from build123d import *

# Parameters (mm, degrees)
SKETCH1_R           = 40
BOSS_EXTRUDE1_DEPTH = 16
CUT_EXTRUDE2_DEPTH  = 500


with BuildPart() as part:
    # Sketch1 → Boss-Extrude1 (new body)
    with BuildSketch(Plane.XY):
        with BuildLine():
            Line((0, 40), (0, 164))
            Line((0, 164), (489.6, 105))
            Line((489.6, 105), (489.6, 40))
            ThreePointArc((489.6, 40), (449.6, 0), (489.6, -40))
            Line((489.6, -40), (489.6, -105))
            Line((489.6, -105), (0, -164))
            Line((0, -164), (0, -40))
            ThreePointArc((0, -40), (40, 0), (0, 40))
        make_face()
        with Locations((241.4, 0)):
            Circle(SKETCH1_R, mode=Mode.SUBTRACT)
        with Locations((126.4, 88.333889345)):
            Circle(SKETCH1_R, mode=Mode.SUBTRACT)
        with Locations((356.4, 60.617386077)):
            Circle(SKETCH1_R, mode=Mode.SUBTRACT)
        with Locations((126.4, -88.333889345)):
            Circle(SKETCH1_R, mode=Mode.SUBTRACT)
        with Locations((356.4, -60.617386077)):
            Circle(SKETCH1_R, mode=Mode.SUBTRACT)
    extrude(amount=BOSS_EXTRUDE1_DEPTH)

    # Sketch3 → Cut-Extrude2 (cut, along a direction that is not the sketch's normal)
    with BuildSketch(Plane(origin=(19.480184067, -161.652510498, 0), x_dir=(0.9928172236743598, 0.11964096445422229, 0), z_dir=(0.11964096445422229, -0.9928172236743598, 0))):
        Polygon((473.521011443, 16), (464.021011443, 0), (473.521011443, 0), align=None)
        Polygon((-19.62111817, 16), (-19.62111817, 0), (13.87888183, 0), align=None)
    extrude(amount=-CUT_EXTRUDE2_DEPTH, dir=(0, -1, 0), mode=Mode.SUBTRACT)


solid = part.part
The listing builds one solid part. Answer for the finished solid, in the listing's coordinates (mm). Round coordinates to 2 decimals unless told otherwise and drop trailing zeros. Write each loop counter-clockwise with the first axis right and the second up, starting at its lowest first coordinate (ties: lowest second). Pieces come first, ordered by that corner, then holes. Notation, with made-up numbers: (18, -24.75) - (47, -24.75) arc R17 cw to (47, -9.75) - close; hole circle Ø3 at (9.25, 66.25). An arc over 180 degrees is marked (long way). Use one line per item in the form item = value. Start each with the question number.
Item 1: A cutting plane is placed at C-C (x = 356.4). Write down the section's boundary in (y, z).
Item 2: Determine the mould class of faces 1 (the flat face through (248.227, -134.087, 7.888)), 2 (the flat face through (17.05, -94.02, 7.8)), 3 (the flat face through (241.373, 134.913, 7.888)), 4 (the cylindrical face through (279.553, 12.015, 7.888)) for opening direction Y: +Y half, -Y half, draft (parallel to the pull), parting line (faces both ways), or undercut.
Item 3: Flat-ended cylindrical pins translate along their axes: pin 1 Ø3 at (y, z) = (-54.5, 10) entering from -X; pin 2 Ø5 at (x, z) = (75, 3) entering from -Y; pin 3 Ø1 at (y, z) = (-17, 6.5) entering from +X. Find the tip coordinate at first contact, or state that the pin passes through.
Item 4: A cutting plane is placed at B-B (y = -55.5). Write down the section's boundary in (x, z), plus the area to 3 significant figures.
Item 5: A cutting plane is placed at A-A (x = 269). Write down the section's boundary in (y, z), plus the area to 3 significant figures.
Item 6: Find the intervals of material crossed by line 1 (X direction, y = 73, z = 5.75); line 2 (X direction, y = -61, z = 10.5); line 3 (Y direction, x = 126.4, z = 4.25), in increasing order. Write a range as [from, to].
Item 7: A cutting plane is placed at D-D (z = 7.25). Write down the section's boundary in (x, y), plus the area to 3 significant figures.
The answers:
q1.outline = (-121.05, 0) - (-100.62, 0) - (-100.62, 16) - (-121.05, 16) - close; (-20.62, 0) - (20.62, 0) - (20.62, 16) - (-20.62, 16) - close; (100.62, 0) - (121.05, 0) - (121.05, 16) - (100.62, 16) - close
q2.face_1 = -Y half
q2.face_2 = draft
q2.face_3 = +Y half
q2.face_4 = undercut
q3.pin_1 = 9.35
q3.pin_2 = -155.26
q3.pin_3 = 453.63
q4.outline = (0, 16) - (33.26, 0) - (103.55, 0) - (103.55, 16) - close; (149.25, 0) - (316.73, 0) - (316.73, 16) - (149.25, 16) - close; (396.07, 0) - (480.17, 0) - (489.6, 16) - (396.07, 16) - close
q4.area = 5,490 mm^2
q5.outline = (-131.58, 0) - (-28.95, 0) - (-28.95, 16) - (-131.58, 16) - close; (28.95, 0) - (131.58, 0) - (131.58, 16) - (28.95, 16) - close
q5.area = 3,280 mm^2
q6.line_1 = [21.31, 89.46], [163.34, 318.36], [394.44, 483.56]
q6.line_2 = [11.43, 97.2], [155.6, 316.4], [396.4, 486.36]
q6.line_3 = [-148.77, -128.33], [-48.33, 48.33], [128.33, 148.77]
q7.outline = (18.19, -161.81) - (484.44, -105.62) - (484.44, -39.67) arc R40 cw to (484.44, 39.67) - (484.44, 105.62) - (18.19, 161.81) - (18.19, 35.63) arc R40 cw to (18.19, -35.63) - close; hole circle Ø80 at (126.4, -88.33); hole circle Ø80 at (126.4, 88.33); hole circle Ø80 at (241.4, 0); hole circle Ø80 at (356.4, -60.62); hole circle Ø80 at (356.4, 60.62)
q7.area = 96,300 mm^2
